from build123d import *

# Parameters (mm, degrees)
SKETCH_1_W                = 20
SKETCH_1_H                = 25
EXTRUDE_1_DEPTH           = 223
HOLE_WIZARD_1_D           = 9
HOLE_WIZARD_1_CBORE_D     = 15
HOLE_WIZARD_1_CBORE_DEPTH = 9
PATTERN_LINEAR_1_COUNT    = 3
PATTERN_LINEAR_1_PITCH    = 50
SKETCH_6_W                = 20
SKETCH_6_H                = 50
EXTRUDE_3_DEPTH           = 70
SKETCH_7_W                = 20
SKETCH_7_H                = 130
EXTRUDE_4_DEPTH           = 30
HOLE_WIZARD_M16_1_D       = 14
HOLE_WIZARD_M16_1_DEPTH   = 38
HOLE_WIZARD_M16_1_TIP     = 4.206024333
CHAMFER_1_SIZE            = 5
FILLET_1_R                = 10
CHAMFER_2_SIZE            = 5


with BuildPart() as part:
    # 草图1 → 凸台-拉伸1 (new body)
    with BuildSketch(Plane.XY):
        Rectangle(SKETCH_1_W, SKETCH_1_H)
    extrude(amount=EXTRUDE_1_DEPTH)

    # 打孔尺寸(%根据)内六角圆柱头螺钉的类型1 (through all)
    with Locations(Plane(origin=(0, 12.5, 0), x_dir=(1, 0, 0), z_dir=(0, 1, 0))):
        with Locations((0, -20)):
            hole_wizard_1 = CounterBoreHole(HOLE_WIZARD_1_D / 2, HOLE_WIZARD_1_CBORE_D / 2, HOLE_WIZARD_1_CBORE_DEPTH)

    # 阵列(线性)1: 打孔尺寸(%根据)内六角圆柱头螺钉的类型1 ×3
    with Locations(*[(0, 0, i * PATTERN_LINEAR_1_PITCH) for i in range(1, PATTERN_LINEAR_1_COUNT)]):
        add(hole_wizard_1, mode=Mode.SUBTRACT)

    # 草图6 → 凸台-拉伸3 (add)
    with BuildSketch(Plane(origin=(0, 12.5, 0), x_dir=(1, 0, 0), z_dir=(0, 1, 0))):
        with Locations((0, -198)):
            Rectangle(SKETCH_6_W, SKETCH_6_H)
    extrude(amount=EXTRUDE_3_DEPTH)

    # 草图7 → 凸台-拉伸4 (add)
    with BuildSketch(Plane(origin=(0, 82.5, 0), x_dir=(1, 0, 0), z_dir=(0, 1, 0))):
        with Locations((0, -158)):
            Rectangle(SKETCH_7_W, SKETCH_7_H)
    extrude(amount=EXTRUDE_4_DEPTH)

    # M16 螺纹孔1
    with Locations(Plane(origin=(0, 112.5, 0), x_dir=(1, 0, 0), z_dir=(0, 1, 0))):
        with Locations((0, -113)):
            Hole(HOLE_WIZARD_M16_1_D / 2, depth=HOLE_WIZARD_M16_1_DEPTH)
            with Locations((0, 0, -(HOLE_WIZARD_M16_1_DEPTH + HOLE_WIZARD_M16_1_TIP / 2))):  # 118° drill point
                Cone(0, HOLE_WIZARD_M16_1_D / 2, HOLE_WIZARD_M16_1_TIP, mode=Mode.SUBTRACT)

    # 倒角1
    chamfer_1_edges = [part.edges().sort_by_distance(p)[0] for p in [
        (0, 82.5, 93),
        (0, 112.5, 93),
    ]]
    chamfer(chamfer_1_edges, length=CHAMFER_1_SIZE)

    # 圆角1
    fillet_1_edges = [part.edges().sort_by_distance(p)[0] for p in [
        (0, 12.5, 173),
        (0, 82.5, 173),
    ]]
    fillet(fillet_1_edges, radius=FILLET_1_R)

    # 倒角2
    chamfer_2_edges = [part.edges().sort_by_distance(p)[0] for p in [
        (0, -12.5, 223),
        (0, 112.5, 223),
    ]]
    chamfer(chamfer_2_edges, length=CHAMFER_2_SIZE)


solid = part.part
Check sheet for the modelled part. Datum: model origin and axes. Units: mm. A direction names the side the tool comes from. Give positions to 0.01 mm unless a question says otherwise; leave off trailing zeros. Loops run counter-clockwise (first coordinate to the right, second up) from the corner with the lowest first, then second, coordinate; pieces in that order, holes last. Notation, with made-up numbers: M -20.75,82 L 30.25,82 A29 ccw 30.25,116 Z; hole C 39.25,51 d2. An arc over 180 degrees is marked long. Return JSON: item names as keys, results as strings. Group by question number.
1. Cross-section at A-A on z = 138.5. Record the boundary of the cut face in (x, y).
2. Cross-section at D-D on z = 20. Record the boundary of the cut face in (x, y).
3. Cross-section at C-C on y = 7. Record the boundary of the cut face in (x, z).
4. Thickness scan on L1, parallel to Z at x = 0, y = 10.5; L2, parallel to Z at x = 0, y = 0.5; L3, parallel to Y at x = 0.5, z = 152.5. Record the ranges inside material, lowest first.
5. Mould release check, pull along Z, two halves, no side actions. Record for faces 4 (the cylindrical face through (0.14, 15.35, 169.99)), 5 (the flat face through (-0.1, 110, 220.5)), 6 (the cylindrical face through (0.59, -4.61, 15.54)), 7 (the flat face through (-10, 7, 138)): released by +Z, released by -Z, zero draft, split by the parting line, or undercut.
6. Go/stop test with flat-tipped pins: pin 1 (8 mm diameter, centred on x = 5, y = 93, fed in from -Z); pin 2 (8 mm diameter, centred on x = -6.5, z = 32.5, fed in from +Y); pin 3 (7.5 mm diameter, centred on x = 0, z = 17, fed in from +Y); pin 4 (7.5 mm diameter, centred on x = 3.5, z = 118, fed in from +Y). Record where each tip stops, or that it passes through.
7. Tool access check on faces 1 (the flat face through (-0.1, 85, 95.5)), 2 (the cylindrical face through (3.461, 8.063, 126.654)), 3 (the flat face through (5, 3.5, 20)). Record the directions out of +Z, -Z, +X, -X, +Y, -Y that give a thin tool (end or side, any length) a straight path to the whole face; none if there is none.
8. Cross-section at B-B on y = 97. Record the boundary of the cut face in (x, z), plus the area to 3 significant figures.
Return value:
{
 "1": {"outline": "M -10,-12.5 L 10,-12.5 L 10,12.5 L -10,12.5 Z; M -10,82.5 L 10,82.5 L 10,112.5 L -10,112.5 Z"},
 "2": {"outline": "M -10,-12.5 L -4.5,-12.5 L -4.5,3.5 L -7.5,3.5 L -7.5,12.5 L -10,12.5 Z; M 4.5,-12.5 L 10,-12.5 L 10,12.5 L 7.5,12.5 L 7.5,3.5 L 4.5,3.5 Z"},
 "3": {"outline": "M -10,0 L 10,0 L 10,223 L -10,223 Z; hole C 0,20 d15; hole C 0,70 d15; hole C 0,120 d15"},
 "4": {"L1": "0 to 12.5, 27.5 to 62.5, 77.5 to 112.5, 127.5 to 223", "L2": "0 to 15.5, 24.5 to 65.5, 74.5 to 115.5, 124.5 to 223", "L3": "-12.5 to 12.5, 82.5 to 112.5"},
 "5": {"face 4": "released by -Z", "face 5": "released by +Z", "face 6": "undercut", "face 7": "zero draft"},
 "6": {"pin 1": "z = 93", "pin 2": "y = 12.5", "pin 3": "y = 3.5", "pin 4": "y = 112.5"},
 "7": {"face 1": "-Z, +X, -X", "face 2": "none", "face 3": "+Y"},
 "8": {"outline": "M -10,93 L 10,93 L 10,223 L -10,223 Z; hole C 0,113 d14", "area": "2,450 mm^2"}
}
